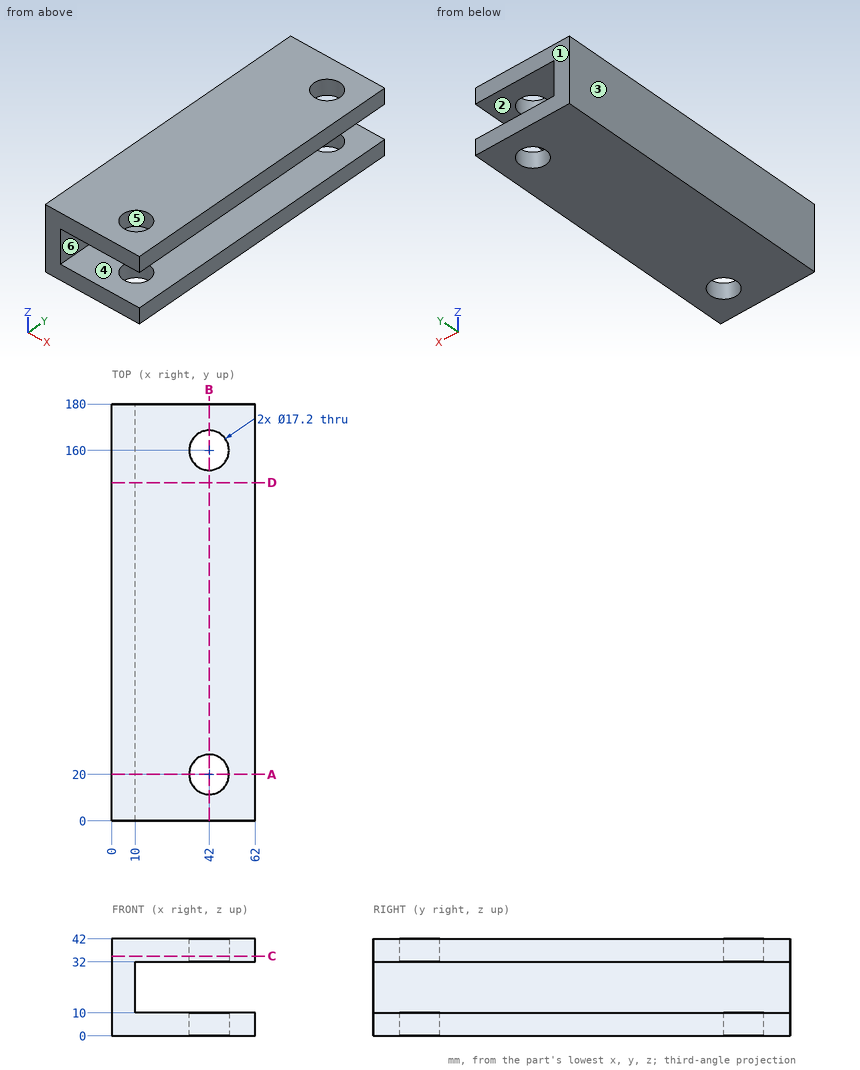
Geometry check sheet. Reference: drawing and pictorial views, mm from the part's lowest x, y, z. A direction names the side the tool comes from. Round coordinates to 2 decimals unless told otherwise and drop trailing zeros. Loops run counter-clockwise (first coordinate to the right, second up) from the corner with the lowest first, then second, coordinate; pieces in that order, holes last. Notation, with made-up numbers: (-21.75, -13.75) - (31.25, -13.75) arc R35 ccw to (31.25, 23.25) - close; hole circle Ø10 at (-21.75, 26). An arc over 180 degrees is marked (long way). Write item = value, one per line. Start each with the question number.
Q1. Thickness scan on L1, parallel to Y at x = 42, z = 2.75; L2, parallel to Z at x = 41, y = 172; L3, parallel to X at y = 108.5, z = 24. Record the ranges inside material, lowest first.
Q2. Section check D-D (y = 146). Record the boundary of the cut face in (x, z).
Q3. Section check B-B (x = 42). Record the boundary of the cut face in (y, z).
Q4. Section check A-A (y = 20). Record the boundary of the cut face in (x, z).
Q5. Section check C-C (z = 34.5). Record the boundary of the cut face in (x, y).
Q6. Release check for a two-part mould opening along X. For the marked faces 3, 4, 5 and 6 record: pulls with the +X half, pulls with the -X half, needs draft (parallel to the pull), parting line crosses it, or undercut.
Q7. Depth check by flat-ended pin: P1, Ø14, axis at x = 42, y = 20, coming from the +Z side; P2, Ø11, axis at y = 133, z = 20.5, coming from the +X side. Enter the tip coordinate at first touch or a pass-through.
Q8. Access from +Z, -Z, +X, -X, +Y, -Y to the whole of each face (thin tool, end or side, straight path). Record for the marked faces 1 and 2.
Derived:
q1.L1 = 0 to 11.4, 28.6 to 151.4, 168.6 to 180
q1.L2 = 0 to 10, 32 to 42
q1.L3 = 0 to 10
q2.outline = (0, 0) - (62, 0) - (62, 10) - (10, 10) - (10, 32) - (62, 32) - (62, 42) - (0, 42) - close
q3.outline = (0, 0) - (11.4, 0) - (11.4, 10) - (0, 10) - close; (0, 32) - (11.4, 32) - (11.4, 42) - (0, 42) - close; (28.6, 0) - (151.4, 0) - (151.4, 10) - (28.6, 10) - close; (28.6, 32) - (151.4, 32) - (151.4, 42) - (28.6, 42) - close; (168.6, 0) - (180, 0) - (180, 10) - (168.6, 10) - close; (168.6, 32) - (180, 32) - (180, 42) - (168.6, 42) - close
q4.outline = (0, 0) - (33.4, 0) - (33.4, 10) - (10, 10) - (10, 32) - (33.4, 32) - (33.4, 42) - (0, 42) - close; (50.6, 0) - (62, 0) - (62, 10) - (50.6, 10) - close; (50.6, 32) - (62, 32) - (62, 42) - (50.6, 42) - close
q5.outline = (0, 0) - (62, 0) - (62, 180) - (0, 180) - close; hole circle Ø17.2 at (42, 20); hole circle Ø17.2 at (42, 160)
q6.face_3 = pulls with the -X half
q6.face_4 = needs draft
q6.face_5 = undercut
q6.face_6 = pulls with the +X half
q7.P1 = through
q7.P2 = 10
q8.face_1 = +Z, -Z, +X, -X, +Y
q8.face_2 = +X, +Y, -Y
